Geometry: final body of the model. Coordinates: model frame, mm. A direction names the side the tool comes from. Round coordinates to 2 decimals unless told otherwise and drop trailing zeros. Loops run counter-clockwise (first coordinate to the right, second up) from the corner with the lowest first, then second, coordinate; pieces in that order, holes last. Notation, with made-up numbers: (74.5, 87) - (129.5, 87) arc R19 cw to (129.5, 110) - close; hole circle Ø3 at (34.5, 83). An arc over 180 degrees is marked (long way). Answer in a Markdown table with one row per item. Add a question column.
from build123d import *

# Parameters (mm, degrees)
LEVER_PLATE_4_4MM_DEPTH             = 4.4
SQUARE_DRIVE_AND_PIN_HOLE_SKETCH_R  = 2.15
SQUARE_DRIVE_AND_PIN_HOLE_CUT_DEPTH = 28.4


with BuildPart() as part:
    # Lever Plate Profile Sketch → Lever Plate 4.4mm (new body)
    with BuildSketch(Plane.XY):
        with BuildLine():
            Line((22.487823695, 6.025594199), (39.772809624, 10.65709222))
            ThreePointArc((39.772809624, 10.65709222), (41.775818518, 12.256700578), (41.962087077, 14.813279454))
            ThreePointArc((41.962087077, 14.813279454), (31.466251763, 31.466251763), (14.813279454, 41.962087077))
            ThreePointArc((14.813279454, 41.962087077), (12.256700578, 41.775818518), (10.65709222, 39.772809624))
            Line((10.65709222, 39.772809624), (6.025594199, 22.487823695))
            ThreePointArc((6.025594199, 22.487823695), (4.720025285, 20.660414916), (2.535022151, 20.14109388))
            ThreePointArc((2.535022151, 20.14109388), (-14.354267658, -14.354267658), (20.14109388, 2.535022151))
            ThreePointArc((20.14109388, 2.535022151), (20.660414916, 4.720025285), (22.487823695, 6.025594199))
        make_face()
    extrude(amount=LEVER_PLATE_4_4MM_DEPTH)

    # Square Drive and Pin Hole Sketch → Square Drive and Pin Hole Cut (cut)
    with BuildSketch(Plane.XY.offset(4.4)):
        with Locations((22.9, 9.5)):
            Circle(SQUARE_DRIVE_AND_PIN_HOLE_SKETCH_R)
        with BuildLine():
            Line((-10.5, 0), (-10.5, -9.5))
            ThreePointArc((-10.5, -9.5), (-10.207106781, -10.207106781), (-9.5, -10.5))
            Line((-9.5, -10.5), (9.5, -10.5))
            ThreePointArc((9.5, -10.5), (10.207106781, -10.207106781), (10.5, -9.5))
            Line((10.5, -9.5), (10.5, 9.5))
            ThreePointArc((10.5, 9.5), (10.207106781, 10.207106781), (9.5, 10.5))
            Line((9.5, 10.5), (-9.5, 10.5))
            ThreePointArc((-9.5, 10.5), (-10.207106781, 10.207106781), (-10.5, 9.5))
            Line((-10.5, 9.5), (-10.5, 0))
        make_face()
    extrude(amount=-SQUARE_DRIVE_AND_PIN_HOLE_CUT_DEPTH, mode=Mode.SUBTRACT)


solid = part.part
1) Material intervals for line 1 along Y through (x, z) = (22.9, 2.85); line 2 along Y through (x, z) = (5, 0.5); line 3 along X through (y, z) = (-13.5, 1.2), sorted ascending. Write a range as from..to.
2) Reachability of faces 1 (the cylindrical face through (12.3, 41.8, 2.2)), 2 (the flat face through (0, -10.5, 2)) from +Z, -Z, +X, -X, +Y, -Y: full face, straight path, thin tool, end or side. Return the list, or none.
3) Pull-direction query (Y, two-part tool) for faces 3 (the flat face through (0, 10.5, 2)), 4 (the cylindrical face through (31.66, 31.27, 2.17)), 5 (the flat face through (10, 11, 0)); classes: pulls with the +Y half, pulls with the -Y half, needs draft (parallel to the pull), parting line crosses it, or undercut.
4) Section C-C, the plane z = 3.55. Return the cut outline in (x, y), and give its area (3 significant figures).
5) Contact query for flat-ended pins moving along their axis: pin 1 Ø2 at (x, z) = (-4, 3) entering from +Y; pin 2 Ø1.5 at (y, z) = (-10.5, 3) entering from +X. Output: stop coordinate, or through.
6) Section A-A, the plane y = 0. Return the cut outline in (x, z), and give its area (3 significant figures).
7) Section D-D, the plane y = 35. Return the cut outline in (x, z), and give its area (3 significant figures).
Evaluation:
| question | item | result |
|---|---|---|
| 1 | line 1 | y = 6.14..7.35, 11.65..38.16 |
| 1 | line 2 | y = -19.67..-10.5, 10.5..20.87 |
| 1 | line 3 | x = -15.16..15.16 |
| 2 | face 1 | +Z, -Z, +Y |
| 2 | face 2 | +Z, -Z |
| 3 | face 3 | undercut |
| 3 | face 4 | pulls with the +Y half |
| 3 | face 5 | needs draft |
| 4 | outline | (2.54, 20.14) arc R20.3 ccw (long way) to (20.14, 2.54) arc R3.2 cw to (22.49, 6.03) - (39.77, 10.66) arc R3.2 ccw to (41.96, 14.81) arc R44.5 ccw to (14.81, 41.96) arc R3.2 ccw to (10.66, 39.77) - (6.03, 22.49) arc R3.2 cw to start; hole (-10.5, -9.5) arc R1 ccw to (-9.5, -10.5) - (9.5, -10.5) arc R1 ccw to (10.5, -9.5) - (10.5, 9.5) arc R1 ccw to (9.5, 10.5) - (-9.5, 10.5) arc R1 ccw to (-10.5, 9.5) - close; hole circle Ø4.3 at (22.9, 9.5) |
| 4 | area | 1,660 mm² |
| 5 | pin 1 | stops at y = 20.08 |
| 5 | pin 2 | stops at x = 17.81 |
| 6 | outline | (-20.3, 0) - (-10.5, 0) - (-10.5, 4.4) - (-20.3, 4.4) - close; (10.5, 0) - (20.3, 0) - (20.3, 4.4) - (10.5, 4.4) - close |
| 6 | area | 86.2 mm² |
| 7 | outline | (9.38, 0) - (27.48, 0) - (27.48, 4.4) - (9.38, 4.4) - close |
| 7 | area | 79.7 mm² |
